Verification items for this drawing (mm, ordinates from the low corner). Coordinates: 2 decimals unless noted, no trailing zeros. Order: outer loops, then holes, each group sorted by start corner. A loop starts at its lowest first (then second) coordinate and runs counter-clockwise, first axis right, second up.
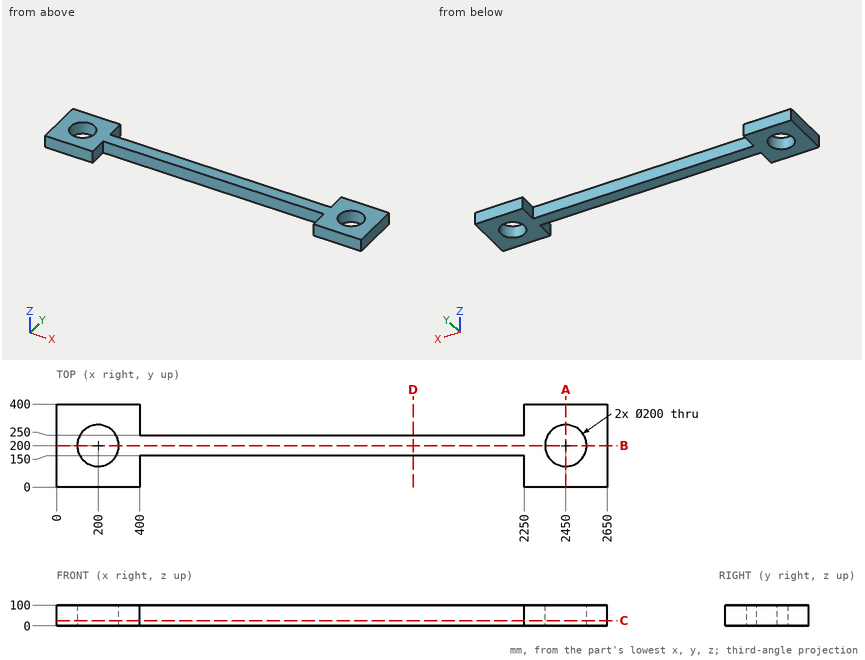
Item 1: Sectioned sample at C-C (z = 25.5). Record the cut outline in (x, y), and give its area (3 significant figures).
Item 2: Sectioned sample at B-B (y = 200). Record the cut outline in (x, z).
Item 3: Sectioned sample at A-A (x = 2450). Record the cut outline in (y, z).
Item 4: Sectioned sample at D-D (x = 1716). Record the cut outline in (y, z), and give its area (3 significant figures).
Item 5: Depth check by flat-ended pin: P1, Ø4, axis at y = 101, z = 56.5, coming from the -X side; P2, Ø8, axis at x = 2025.5, z = 53, coming from the +Y side; P3, Ø8, axis at x = 597, z = 64.5, coming from the -Y side. Enter the tip coordinate at first touch or a pass-through.
Item 6: Thickness scan on line 1 along X through (y, z) = (143, 74); line 2 along X through (y, z) = (96, 95); line 3 along X through (y, z) = (215, 79.5). Record the ranges inside material, lowest first.
Geometry check:
1. outline: (0, 0) - (400, 0) - (400, 150) - (2250, 150) - (2250, 0) - (2650, 0) - (2650, 400) - (2250, 400) - (2250, 250) - (400, 250) - (400, 400) - (0, 400) - close; hole circle Ø200 at (200, 200); hole circle Ø200 at (2450, 200)
1. area: 442,000 mm2
2. outline: (0, 0) - (100, 0) - (100, 100) - (0, 100) - close; (300, 0) - (2350, 0) - (2350, 100) - (300, 100) - close; (2550, 0) - (2650, 0) - (2650, 100) - (2550, 100) - close
3. outline: (0, 0) - (100, 0) - (100, 100) - (0, 100) - close; (300, 0) - (400, 0) - (400, 100) - (300, 100) - close
4. outline: (150, 0) - (250, 0) - (250, 100) - (150, 100) - close
4. area: 10,000 mm2
5. P1: stops at x = 0
5. P2: stops at y = 250
5. P3: stops at y = 150
6. line 1: x = 0 to 117.84, 282.16 to 400, 2250 to 2367.84, 2532.16 to 2650
6. line 2: x = 0 to 400, 2250 to 2650
6. line 3: x = 0 to 101.13, 298.87 to 2351.13, 2548.87 to 2650
